Source: three-view drawing plus pictorial views. Frame: mm from the lowest corner of the part. Give positions to 0.01 mm unless a question says otherwise; leave off trailing zeros. Write each loop counter-clockwise with the first axis right and the second up, starting at its lowest first coordinate (ties: lowest second). Pieces come first, ordered by that corner, then holes.
Q1. Line query: L1, parallel to Y at x = 13.6, z = 1.5; L2, parallel to X at y = 23.5, z = 5.6. Output: solid intervals per line, ascending.
Q2. Cut plane A-A on x = 13.6. Return the cut outline in (y, z), plus the area to 3 significant figures.
Q3. Cut plane B-B on y = 19.65. Return the cut outline in (x, z), plus the area to 3 significant figures.
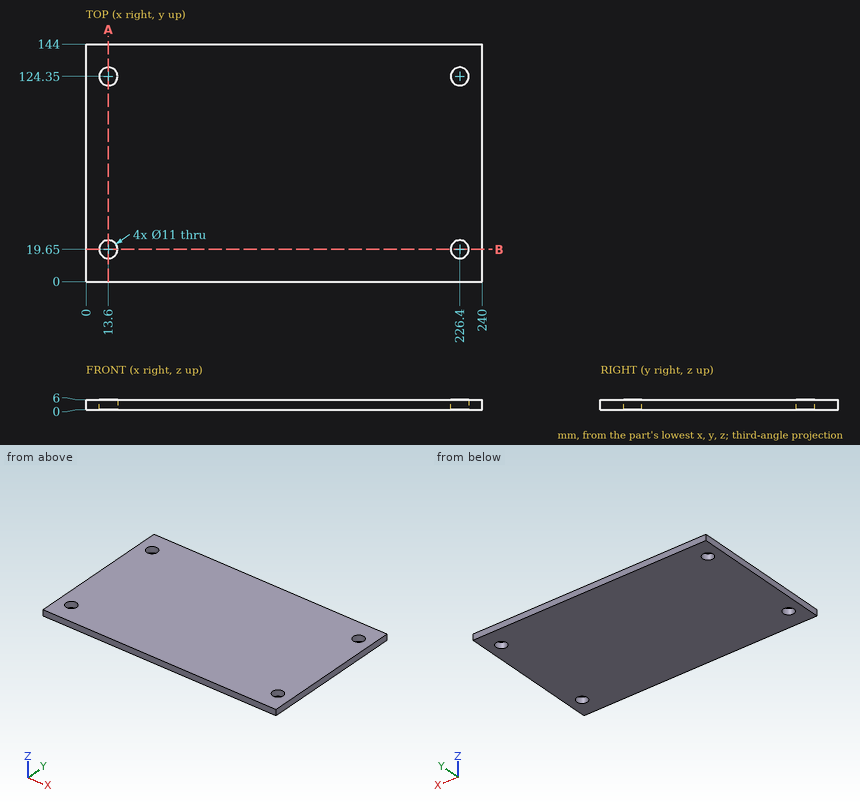
Data:
1. L1: y = 0 to 14.15, 25.15 to 118.85, 129.85 to 144
1. L2: x = 0 to 9.67, 17.53 to 222.47, 230.33 to 240
2. outline: (0, 0) - (14.15, 0) - (14.15, 6) - (0, 6) - close; (25.15, 0) - (118.85, 0) - (118.85, 6) - (25.15, 6) - close; (129.85, 0) - (144, 0) - (144, 6) - (129.85, 6) - close
2. area: 732 mm2
3. outline: (0, 0) - (8.1, 0) - (8.1, 6) - (0, 6) - close; (19.1, 0) - (220.9, 0) - (220.9, 6) - (19.1, 6) - close; (231.9, 0) - (240, 0) - (240, 6) - (231.9, 6) - close
3. area: 1,310 mm2
